from build123d import *

# Parameters (mm, degrees)
BOSS_EXTRUDE1_DEPTH = 100
SKETCH2_R           = 7
BOSS_EXTRUDE2_DEPTH = 3
CHAMFER1_SIZE       = 1
CHAMFER1_SIZE2      = 1.732050808


with BuildPart() as part:
    # Sketch1 → Boss-Extrude1 (new body)
    with BuildSketch(Plane.XY):
        Polygon((2.65, -4.58993464), (5.3, 0), (2.65, 4.58993464), (-2.65, 4.58993464), (-5.3, 0), (-2.65, -4.58993464), align=None)
    extrude(amount=BOSS_EXTRUDE1_DEPTH)

    # Sketch2 → Boss-Extrude2 (add)
    with BuildSketch(Plane(origin=(0, 0, 0), x_dir=(-1, 0, 0), z_dir=(0, 0, -1))):
        Circle(SKETCH2_R)
    extrude(amount=BOSS_EXTRUDE2_DEPTH)

    # Chamfer1
    chamfer1_edges = [part.edges().sort_by_distance(p)[0] for p in [
        (7, 0, -3),
    ]]
    chamfer1_side = [part.faces().sort_by_distance(p)[0] for p in [
        (7, 0, -1.5),
    ]]
    chamfer(chamfer1_edges, length=CHAMFER1_SIZE, length2=CHAMFER1_SIZE2, reference=chamfer1_side[0])


solid = part.part
Read the model definition and answer for the solid it produces. Units are mm, in the model's axes. A direction names the side the tool comes from. Give positions to 0.01 mm unless a question says otherwise; leave off trailing zeros. Write each loop counter-clockwise with the first axis right and the second up, starting at its lowest first coordinate (ties: lowest second). Pieces come first, ordered by that corner, then holes. Notation, with made-up numbers: (34.25, 85) - (78.25, 85) arc R15 ccw to (78.25, 95) - close; hole circle Ø10 at (-8, 76.5). An arc over 180 degrees is marked (long way). Answer in a Markdown table with one row per item. Add a question column.
Item 1: Flat-ended cylindrical pins translate along their axes: P1, Ø3, axis at x = 0.5, z = 44, coming from the +Y side; P2, Ø3, axis at x = -2.5, y = 5, coming from the +Z side; P3, Ø1.5, axis at x = 5.5, y = -4, coming from the +Z side; P4, Ø8, axis at y = 5, z = 64, coming from the -X side. Find the tip coordinate at first contact, or state that the pin passes through.
Item 2: A tool of negligible diameter and unlimited length cuts with its end or side. For faces 1 (the face through (-3.956, 2.327, 49.3)), 2 (the face through (0, -4.59, 49)), 3 (the face through (-5, 2, 0)), from which of +Z, -Z, +X, -X, +Y, -Y can it reach the whole face along a straight path? Write none if from no direction.
Item 3: Section A-A, the plane x = 0 is taken. Write down the section's boundary in (y, z), and give its area (3 significant figures).
Item 4: Section B-B, the plane z = 62 is taken. Write down the section's boundary in (x, y).
Item 5: Find the intervals of material crossed by L1, parallel to Y at x = -1, z = 37; L2, parallel to Z at x = -3.25, y = 3.75; L3, parallel to Y at x = 4.5, z = 37, in increasing order.
Recorded:
| question | item | result |
|---|---|---|
| 1 | P1 | stops at y = 4.59 |
| 1 | P2 | stops at z = 100 |
| 1 | P3 | stops at z = 0 |
| 1 | P4 | stops at x = -4.72 |
| 2 | face 1 | +Z, -X, +Y |
| 2 | face 2 | +Z, +X, -X, -Y |
| 2 | face 3 | +Z |
| 3 | outline | (-7, -2) - (-5.27, -3) - (5.27, -3) - (7, -2) - (7, 0) - (4.59, 0) - (4.59, 100) - (-4.59, 100) - (-4.59, 0) - (-7, 0) - close |
| 3 | area | 958 mm2 |
| 4 | outline | (-5.3, 0) - (-2.65, -4.59) - (2.65, -4.59) - (5.3, 0) - (2.65, 4.59) - (-2.65, 4.59) - close |
| 5 | L1 | y = -4.59 to 4.59 |
| 5 | L2 | z = -3 to 0 |
| 5 | L3 | y = -1.39 to 1.39 |
